Check sheet for the modelled part. Datum: model origin and axes. Units: mm. A direction names the side the tool comes from. Coordinates: 2 decimals unless noted, no trailing zeros. Loops run counter-clockwise (first coordinate to the right, second up) from the corner with the lowest first, then second, coordinate; pieces in that order, holes last. Notation, with made-up numbers: (9.5, -37) - (25.5, -37) arc R36 ccw to (25.5, -1) - close; hole circle Ø9 at (-14, 67.5). An arc over 180 degrees is marked (long way). Use a Markdown table: item, result. Add a question column.
1) Thickness scan on line 1 (Z direction, x = -23, y = 113); line 2 (Y direction, x = -21.25, z = -31); line 3 (Y direction, x = -26, z = -24). Record the ranges inside material, lowest first.
2) Sectioned sample at A-A, the plane y = 71. Enter the section's corners in (x, z), then the cut area to 3 significant figures.
3) Go/stop test with flat-tipped pins: P1, Ø16, axis at x = -17, z = -19, coming from the +Y side; P2, Ø3, axis at x = -19, z = 27.5, coming from the +Y side; P3, Ø5.5, axis at y = 22, z = 16, coming from the -X side; P4, Ø2, axis at y = 116.5, z = -22, coming from the -X side. Record where each tip stops, or that it passes through.
4) Sectioned sample at B-B, the plane y = 90. Enter the section's corners in (x, z), then the cut area to 3 significant figures.
5) Sectioned sample at D-D, the plane x = -12.5. Enter the section's corners in (y, z) (3 decimals), then the cut area to 3 significant figures.
6) Sectioned sample at C-C, the plane x = -23.75. Enter the section's corners in (y, z).
7) Tool access check on faces 4 (the flat face through (-20, 101, 11)), 5 (the cylindrical face through (-24.93, 127.5, 27.34)), 6 (the flat face through (0, 18, 1)), 7 (the flat face through (-22, 48, -47.5)), 8 (the flat face through (-10, 21, 1)). Record the directions out of +Z, -Z, +X, -X, +Y, -Y that give a thin tool (end or side, any length) a straight path to the whole face; none if there is none.
8) Draft check along Y on faces 1 (the flat face through (-22, 48, 47.5)), 2 (the flat face through (-25, 113, 7.5)), 3 (the cylindrical face through (-24.93, 141.34, -21.92)). Enter one of: pulls with the +Y half, pulls with the -Y half, needs draft (parallel to the pull), parting line crosses it, or undercut.
from build123d import *

# Parameters (mm, degrees)
SUPPORT_BODY_DEPTH         = 47.5
MOUNTING_SLOTS_3X7MM_REACH = 170.096


with BuildPart() as part:
    # Support Profile Sketch → Support Body (new, symmetric)
    with BuildSketch(Plane.XY):
        Polygon((-30, 0), (0, 0), (0, 37.09481005), (-20, 44.09481005), (-20, 160), (-30, 160), (-30, 37), (-10, 30), (-10, 12), (-30, 12), align=None)
    extrude(amount=SUPPORT_BODY_DEPTH, both=True)

    # Mounting Slots Sketch → Mounting Slots 3x7mm (cut, up to next)
    with BuildSketch(Plane(origin=(-20, 0, 0), x_dir=(0, 0, -1), z_dir=(1, 0, 0)), mode=Mode.PRIVATE) as mounting_slots_3x7mm_sk1:
        with BuildLine():
            Line((-35, 120), (-35, 65))
            ThreePointArc((-35, 65), (-27.5, 57.5), (-20, 65))
            Line((-20, 65), (-20, 120))
            ThreePointArc((-20, 120), (-27.5, 127.5), (-35, 120))
        make_face()
    mounting_slots_3x7mm_tool1 = extrude(mounting_slots_3x7mm_sk1.sketch, amount=-MOUNTING_SLOTS_3X7MM_REACH, mode=Mode.PRIVATE) & part.part
    # Mounting Slots Sketch → Mounting Slots 3x7mm (cut, up to next)
    with BuildSketch(Plane(origin=(-20, 0, 0), x_dir=(0, 0, -1), z_dir=(1, 0, 0)), mode=Mode.PRIVATE) as mounting_slots_3x7mm_sk2:
        with BuildLine():
            Line((-7.5, 140), (-7.5, 85))
            ThreePointArc((-7.5, 85), (0, 77.5), (7.5, 85))
            Line((7.5, 85), (7.5, 140))
            ThreePointArc((7.5, 140), (0, 147.5), (-7.5, 140))
        make_face()
    mounting_slots_3x7mm_tool2 = extrude(mounting_slots_3x7mm_sk2.sketch, amount=-MOUNTING_SLOTS_3X7MM_REACH, mode=Mode.PRIVATE) & part.part
    # Mounting Slots Sketch → Mounting Slots 3x7mm (cut, up to next)
    with BuildSketch(Plane(origin=(-20, 0, 0), x_dir=(0, 0, -1), z_dir=(1, 0, 0)), mode=Mode.PRIVATE) as mounting_slots_3x7mm_sk3:
        with BuildLine():
            ThreePointArc((35, 65), (27.5, 57.5), (20, 65))
            Line((20, 65), (20, 120))
            ThreePointArc((20, 120), (27.5, 127.5), (35, 120))
            Line((35, 120), (35, 65))
        make_face()
    mounting_slots_3x7mm_tool3 = extrude(mounting_slots_3x7mm_sk3.sketch, amount=-MOUNTING_SLOTS_3X7MM_REACH, mode=Mode.PRIVATE) & part.part
    # Mounting Slots Sketch → Mounting Slots 3x7mm (cut, up to next)
    with BuildSketch(Plane(origin=(-20, 0, 0), x_dir=(0, 0, -1), z_dir=(1, 0, 0)), mode=Mode.PRIVATE) as mounting_slots_3x7mm_sk4:
        with BuildLine():
            ThreePointArc((26.453123952, 139.97258247), (41.267034521, 134.507541504), (47.5, 120))
            Line((47.5, 120), (47.5, 160))
            Line((47.5, 160), (1.13e-07, 160))
            ThreePointArc((1.13e-07, 160), (12.182870127, 155.861200316), (19.323494322, 145.157767656))
            ThreePointArc((19.323494322, 145.157767656), (21.969515451, 141.301833745), (26.453123952, 139.97258247))
        make_face()
    mounting_slots_3x7mm_tool4 = extrude(mounting_slots_3x7mm_sk4.sketch, amount=-MOUNTING_SLOTS_3X7MM_REACH, mode=Mode.PRIVATE) & part.part
    # Mounting Slots Sketch → Mounting Slots 3x7mm (cut, up to next)
    with BuildSketch(Plane(origin=(-20, 0, 0), x_dir=(0, 0, -1), z_dir=(1, 0, 0)), mode=Mode.PRIVATE) as mounting_slots_3x7mm_sk5:
        with BuildLine():
            ThreePointArc((-19.323494322, 145.157767656), (-12.182870037, 155.861200385), (1.13e-07, 160))
            Line((1.13e-07, 160), (-47.5, 160))
            Line((-47.5, 160), (-47.5, 120))
            ThreePointArc((-47.5, 120), (-41.267034521, 134.507541504), (-26.453123952, 139.97258247))
            ThreePointArc((-26.453123952, 139.97258247), (-21.969515451, 141.301833745), (-19.323494322, 145.157767656))
        make_face()
    mounting_slots_3x7mm_tool5 = extrude(mounting_slots_3x7mm_sk5.sketch, amount=-MOUNTING_SLOTS_3X7MM_REACH, mode=Mode.PRIVATE) & part.part
    add(mounting_slots_3x7mm_tool1.solids().sort_by_distance((-20, 92.5, 27.5))[0], mode=Mode.SUBTRACT)
    add(mounting_slots_3x7mm_tool2.solids().sort_by_distance((-20, 112.5, 0))[0], mode=Mode.SUBTRACT)
    add(mounting_slots_3x7mm_tool3.solids().sort_by_distance((-20, 92.5, -27.5))[0], mode=Mode.SUBTRACT)
    add(mounting_slots_3x7mm_tool4.solids().sort_by_distance((-20, 149.008344, -32.791963))[0], mode=Mode.SUBTRACT)
    add(mounting_slots_3x7mm_tool5.solids().sort_by_distance((-20, 149.008344, 32.791963))[0], mode=Mode.SUBTRACT)


solid = part.part
Solved:
| question | item | result |
|---|---|---|
| 1 | line 1 | z = -47.5 to -35, -20 to -7.5, 7.5 to 20, 35 to 47.5 |
| 1 | line 2 | y = 0 to 12, 33.94 to 58.37, 126.63 to 139.69 |
| 1 | line 3 | y = 0 to 12, 35.6 to 58.37, 126.63 to 140.28 |
| 2 | outline | (-30, -47.5) - (-20, -47.5) - (-20, -35) - (-30, -35) - close; (-30, -20) - (-20, -20) - (-20, 20) - (-30, 20) - close; (-30, 35) - (-20, 35) - (-20, 47.5) - (-30, 47.5) - close |
| 2 | area | 650 mm2 |
| 3 | P1 | stops at y = 156.3 |
| 3 | P2 | stops at y = 140 |
| 3 | P3 | stops at x = -10 |
| 3 | P4 | passes through |
| 4 | outline | (-30, -47.5) - (-20, -47.5) - (-20, -35) - (-30, -35) - close; (-30, -20) - (-20, -20) - (-20, -7.5) - (-30, -7.5) - close; (-30, 7.5) - (-20, 7.5) - (-20, 20) - (-30, 20) - close; (-30, 35) - (-20, 35) - (-20, 47.5) - (-30, 47.5) - close |
| 4 | area | 500 mm2 |
| 5 | outline | (0, -47.5) - (12, -47.5) - (12, 47.5) - (0, 47.5) - close; (30.875, -47.5) - (41.47, -47.5) - (41.47, 47.5) - (30.875, 47.5) - close |
| 5 | area | 2,150 mm2 |
| 6 | outline | (0, -47.5) - (12, -47.5) - (12, 47.5) - (0, 47.5) - close; (34.81, -47.5) - (120, -47.5) arc R20 ccw to (139.97, -26.45) arc R7 cw to (145.16, -19.32) arc R20 ccw to (145.16, 19.32) arc R7 cw to (139.97, 26.45) arc R20 ccw to (120, 47.5) - (34.81, 47.5) - close; hole (65, -35) - (120, -35) arc R7.5 ccw to (120, -20) - (65, -20) arc R7.5 ccw to start; hole (65, 20) - (120, 20) arc R7.5 ccw to (120, 35) - (65, 35) arc R7.5 ccw to start; hole (85, -7.5) - (140, -7.5) arc R7.5 ccw to (140, 7.5) - (85, 7.5) arc R7.5 ccw to start |
| 7 | face 4 | +Z, -Z, +X, +Y |
| 7 | face 5 | +X, -X |
| 7 | face 6 | +Z, -Z, +X, +Y, -Y |
| 7 | face 7 | -Z, +X, -X, +Y, -Y |
| 7 | face 8 | +Z, -Z, -X |
| 8 | face 1 | needs draft |
| 8 | face 2 | undercut |
| 8 | face 3 | pulls with the +Y half |
